Part model, mm, in its own coordinate system. A direction names the side the tool comes from. Give positions to 0.01 mm unless a question says otherwise; leave off trailing zeros. Order: outer loops, then holes, each group sorted by start corner. A loop starts at its lowest first (then second) coordinate and runs counter-clockwise, first axis right, second up. Notation, with made-up numbers: M 16.25,72.25 L 28.25,72.25 A17 cw 28.25,80.25 Z; hole C -25,52 d1. An arc over 180 degrees is marked long. One line per question, with ' | ' between items.
```python
from build123d import *

# Parameters (mm, degrees)
SKETCH_1_W             = 65
SKETCH_1_H             = 37
EXTRUDE_1_DEPTH        = 8
SKETCH_3_W             = 32
SKETCH_3_H             = 29
CUT_EXTRUDE_1_DEPTH    = 41.675545479
HOLE_WIZARD_M6_1_D     = 5
HOLE_WIZARD_M8_2_D     = 6.8
HOLE_WIZARD_M8_2_DEPTH = 22.25
HOLE_WIZARD_M8_2_TIP   = 2.042926105
CHAMFER_1_SIZE         = 2


with BuildPart() as part:
    # 草图1 → 凸台-拉伸1 (new, symmetric)
    with BuildSketch(Plane.XY):
        Rectangle(SKETCH_1_W, SKETCH_1_H)
    extrude(amount=EXTRUDE_1_DEPTH, both=True)

    # 草图3 → 切除-拉伸1 (cut, through all)
    with BuildSketch(Plane.XY.offset(8)):
        with Locations((0, -4)):
            Rectangle(SKETCH_3_W, SKETCH_3_H)
    extrude(amount=-CUT_EXTRUDE_1_DEPTH, mode=Mode.SUBTRACT)

    # M6 螺纹孔1 (through all)
    with Locations(Plane(origin=(32.5, 0, 0), x_dir=(0, 0, -1), z_dir=(1, 0, 0))):
        with Locations((0, -10)):
            Hole(HOLE_WIZARD_M6_1_D / 2)

    # M8 螺纹孔2
    with Locations(Plane(origin=(0, 18.5, 0), x_dir=(1, 0, 0), z_dir=(0, 1, 0))):
        with Locations((-22.5, 0), (22.5, 0)):
            Hole(HOLE_WIZARD_M8_2_D / 2, depth=HOLE_WIZARD_M8_2_DEPTH)
            with Locations((0, 0, -(HOLE_WIZARD_M8_2_DEPTH + HOLE_WIZARD_M8_2_TIP / 2))):  # 118° drill point
                Cone(0, HOLE_WIZARD_M8_2_D / 2, HOLE_WIZARD_M8_2_TIP, mode=Mode.SUBTRACT)

    # 倒角1
    chamfer_1_edges = [part.edges().sort_by_distance(p)[0] for p in [
        (24.25, -18.5, -8),
        (24.25, -18.5, 8),
        (-24.25, -18.5, -8),
        (-24.25, -18.5, 8),
    ]]
    chamfer(chamfer_1_edges, length=CHAMFER_1_SIZE)


solid = part.part
```
1. Probe L1, parallel to X at y = 2.5, z = 4.5; L2, parallel to Z at x = -22.5, y = 1.5; L3, parallel to Y at x = -10, z = -1. List the from-to ranges inside material, lowest first. Write a range as from..to.
Worked out:
L1: x = -32.5..-16, 16..32.5 | L2: z = -8..-3.4, 3.4..8 | L3: y = 10.5..18.5
2. Slice it at D-D on y = -10. Give the cut face in (x, z), then the cut area to 3 significant figures.
Worked out:
outline: M -32.5,-8 L -16,-8 L -16,-2.5 L -32.5,-2.5 Z; M -32.5,2.5 L -16,2.5 L -16,8 L -32.5,8 Z; M 16,-8 L 32.5,-8 L 32.5,-2.5 L 16,-2.5 Z; M 16,2.5 L 32.5,2.5 L 32.5,8 L 16,8 Z | area: 363 mm2
3. Slice it at C-C on z = -4.75. Give the cut face in (x, y).
Worked out:
outline: M -32.5,-18.5 L -16,-18.5 L -16,10.5 L 16,10.5 L 16,-18.5 L 32.5,-18.5 L 32.5,18.5 L -32.5,18.5 Z
4. Tool access for faces 1 (the cylindrical face through (24.13, -12.44, -0.54)), 2 (the cylindrical face through (-25.64, 7.22, 1.3)), 3 (the flat face through (16, -4, 0)): list every direction of +Z, -Z, +X, -X, +Y, -Y with a clear straight run to the whole face (end or side of a thin tool).
Worked out:
face 1: +X, -X | face 2: +Y | face 3: +Z, -Z, -Y
5. Drop flat-ended pins along their axis: pin 1 (8 mm diameter, centred on y = -10, z = 0, fed in from +X); pin 2 (12 mm diameter, centred on x = 3, y = 2.5, fed in from -Z); pin 3 (5.5 mm diameter, centred on x = 22.5, z = 0, fed in from +Y); pin 4 (8 mm diameter, centred on x = 2, z = -3, fed in from -Y). Give the stop position or say it passes through.
Worked out:
pin 1: stops at x = 32.5 | pin 2: passes through | pin 3: stops at y = -4.14 | pin 4: stops at y = 10.5
6. Mould opens along Z. For faces 4 (the conical face through (23.06, -5.44, -0.18)), 5 (the flat face through (32.5, 0, 0)), 6 (the flat face through (24.1, -17.5, 7)) say: released by +Z, released by -Z, zero draft, split by the parting line, or undercut.
Worked out:
face 4: undercut | face 5: zero draft | face 6: released by +Z
7. Slice it at B-B on x = 28. Give the cut face in (y, z), then the cut area to 3 significant figures.
Worked out:
outline: M -18.5,-6 L -16.5,-8 L 18.5,-8 L 18.5,8 L -16.5,8 L -18.5,6 Z; hole C -10,0 d5 | area: 568 mm2
8. Slice it at A-A on y = 9.5. Give the cut face in (x, z).
Worked out:
outline: M -32.5,-8 L -16,-8 L -16,8 L -32.5,8 Z; M 16,-8 L 32.5,-8 L 32.5,8 L 16,8 Z; hole C -22.5,0 d6.8; hole C 22.5,0 d6.8
